Part print with two shaded views. Sizes in mm from the minimum x, y, z corner. A direction names the side the tool comes from. Round coordinates to 2 decimals unless told otherwise and drop trailing zeros. Order: outer loops, then holes, each group sorted by start corner. A loop starts at its lowest first (then second) coordinate and runs counter-clockwise, first axis right, second up. Notation, with made-up numbers: (41, 8.25) -> (55, 8.25) arc R21 ccw to (55, 20.25) -> close; hole circle Ø11 at (9, 53.25). An arc over 180 degrees is marked (long way). Put each result on its own line as item: value. Start each with the question number.
Q1. Probe L1, parallel to X at y = 10.75, z = 3; L2, parallel to X at y = 8.5, z = 0.5; L3, parallel to Y at x = 76.5, z = 9.25. List the from-to ranges inside material, lowest first.
Q2. Cut at B-B, the plane z = 5.25. List the corners of the cut face in (x, y).
Q3. Cut at D-D, the plane x = 40.5. List the corners of the cut face in (y, z).
Q4. Flat gauge pins, fed straight in: P1, Ø3, axis at x = 52.5, y = 13.5, coming from the +Z side; P2, Ø2, axis at x = 65.5, y = 9.5, coming from the +Z side. Where does each tip first touch, or does it go through?
Q5. Cut at A-A, the plane x = 65. List the corners of the cut face in (y, z), and give its area (3 significant figures).
Q6. Cut at C-C, the plane y = 16.25. List the corners of the cut face in (x, z), and give its area (3 significant figures).
Q7. 3-axis set-ups, long thin cutter, end or side, ignore diameter. For the marked faces 1 and 2: which of +Z, -Z, +X, -X, +Y, -Y reach the whole face in a straight line?
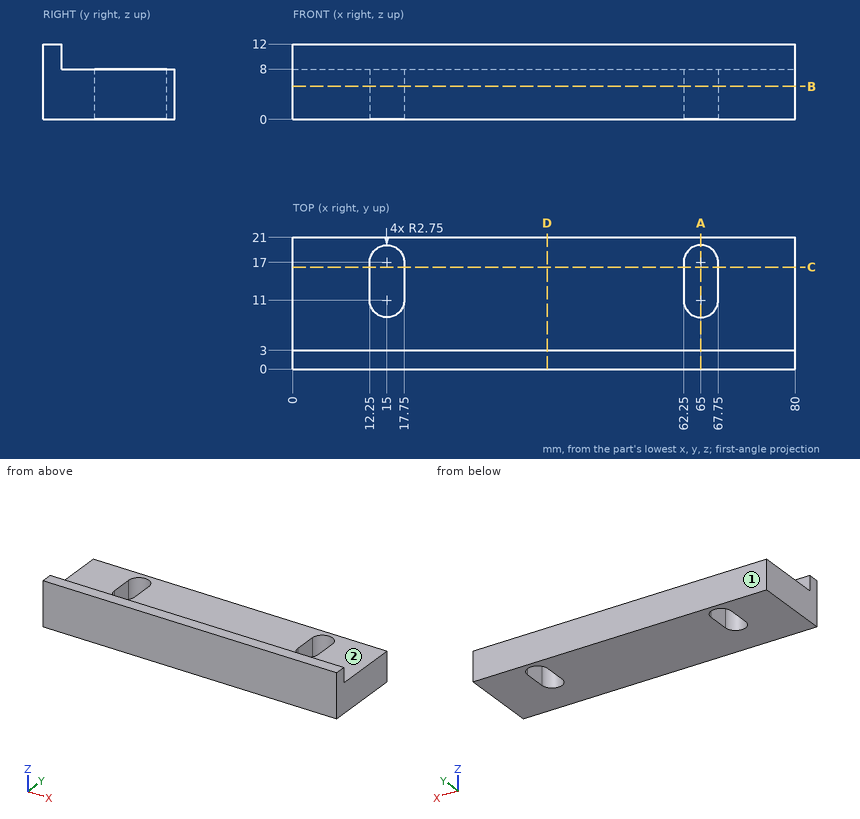
Ans:
1. L1: x = 0 to 12.26, 17.74 to 62.26, 67.74 to 80
1. L2: x = 0 to 13.85, 16.15 to 63.85, 66.15 to 80
1. L3: y = 0 to 3
2. outline: (0, 0) -> (80, 0) -> (80, 21) -> (0, 21) -> close; hole (12.25, 11) arc R2.75 ccw to (17.75, 11) -> (17.75, 17) arc R2.75 ccw to (12.25, 17) -> close; hole (62.25, 11) arc R2.75 ccw to (67.75, 11) -> (67.75, 17) arc R2.75 ccw to (62.25, 17) -> close
3. outline: (0, 0) -> (21, 0) -> (21, 8) -> (3, 8) -> (3, 12) -> (0, 12) -> close
4. P1: stops at z = 8
4. P2: passes through
5. outline: (0, 0) -> (8.25, 0) -> (8.25, 8) -> (3, 8) -> (3, 12) -> (0, 12) -> close; (19.75, 0) -> (21, 0) -> (21, 8) -> (19.75, 8) -> close
5. area: 88.0 mm^2
6. outline: (0, 0) -> (12.25, 0) -> (12.25, 8) -> (0, 8) -> close; (17.75, 0) -> (62.25, 0) -> (62.25, 8) -> (17.75, 8) -> close; (67.75, 0) -> (80, 0) -> (80, 8) -> (67.75, 8) -> close
6. area: 552 mm^2
7. face 1: +Z, -Z, +X, -X, +Y
7. face 2: +Z, +X, -X, +Y
